```python
from build123d import *

# Parameters (mm, degrees)
SKETCH_1_W          = 180
SKETCH_1_H          = 160
EXTRUDE_1_DEPTH     = 5
SKETCH_2_R          = 4
CUT_EXTRUDE_1_DEPTH = 121.519707932


with BuildPart() as part:
    # 草图1 → 凸台-拉伸1 (new body)
    with BuildSketch(Plane.XY):
        Rectangle(SKETCH_1_W, SKETCH_1_H)
    extrude(amount=EXTRUDE_1_DEPTH)

    # 草图2 → 切除-拉伸1 (cut, through all)
    with BuildSketch(Plane.XY.offset(5)):
        with Locations((-65, 65)):
            Circle(SKETCH_2_R)
        with Locations((65, 65)):
            Circle(SKETCH_2_R)
        with Locations((65, -65)):
            Circle(SKETCH_2_R)
        with Locations((-65, -65)):
            Circle(SKETCH_2_R)
    extrude(amount=-CUT_EXTRUDE_1_DEPTH, mode=Mode.SUBTRACT)


solid = part.part
```
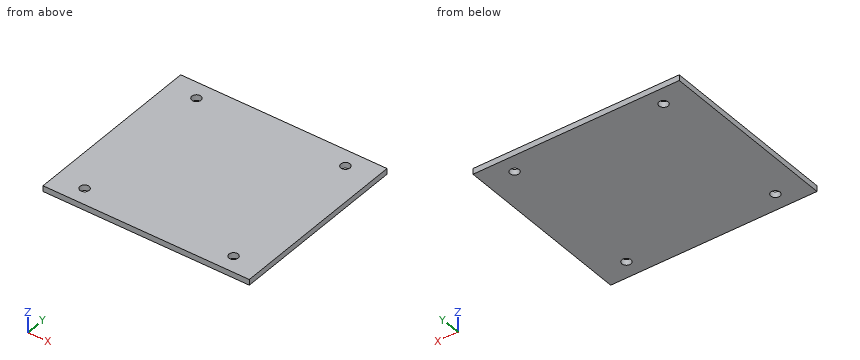
CAD build for the part. Positions are in the model's coordinates, mm. Give positions to 0.01 mm unless a question says otherwise; leave off trailing zeros. Order: outer loops, then holes, each group sorted by start corner. A loop starts at its lowest first (then second) coordinate and runs counter-clockwise, first axis right, second up. Notation, with made-up numbers: M -13.5,-33 L -5.5,-33 A4 cw -5.5,-28 Z; hole C 11,74.25 d5. An arc over 180 degrees is marked long. Put each result on its own line as item: value. Start each with the question number.
(1) Drill centre lines: line 1 along Y through (x, z) = (65, 1.35); line 2 along Y through (x, z) = (-63.5, 2.65); line 3 along X through (y, z) = (-67, 4). Where is each one in solid material? Low to high.
(2) Saw through at B-B, the plane x = -65. Write the cut outline in (y, z).
(3) Saw through at A-A, the plane y = 65. Write the cut outline in (x, z), then the cut area to 3 significant figures.
Check result:
1. line 1: y = -80 to -69, -61 to 61, 69 to 80
1. line 2: y = -80 to -68.71, -61.29 to 61.29, 68.71 to 80
1. line 3: x = -90 to -68.46, -61.54 to 61.54, 68.46 to 90
2. outline: M -80,0 L -69,0 L -69,5 L -80,5 Z; M -61,0 L 61,0 L 61,5 L -61,5 Z; M 69,0 L 80,0 L 80,5 L 69,5 Z
3. outline: M -90,0 L -69,0 L -69,5 L -90,5 Z; M -61,0 L 61,0 L 61,5 L -61,5 Z; M 69,0 L 90,0 L 90,5 L 69,5 Z
3. area: 820 mm2
